```python
from build123d import *

# Parameters (mm, degrees)
BASE_PLATE_SKETCH_R = 7
BASE_PLATE_DEPTH    = 14
PIVOT_LUG_SKETCH_R  = 8
PIVOT_LUG_DEPTH     = 10


with BuildPart() as part:
    # Base Plate Sketch → Base Plate (new body)
    with BuildSketch(Plane.XY):
        with BuildLine():
            Line((-61, 29), (61, 29))
            ThreePointArc((61, 29), (64.535533906, 27.535533906), (66, 24))
            Line((66, 24), (66, -24))
            ThreePointArc((66, -24), (64.535533906, -27.535533906), (61, -29))
            Line((61, -29), (-61, -29))
            ThreePointArc((-61, -29), (-64.535533906, -27.535533906), (-66, -24))
            Line((-66, -24), (-66, 24))
            ThreePointArc((-66, 24), (-64.535533906, 27.535533906), (-61, 29))
        make_face()
        with Locations((-50, 0)):
            Circle(BASE_PLATE_SKETCH_R, mode=Mode.SUBTRACT)
        with Locations(Location((50, 0, 0), (0, 0, 180))):
            Circle(BASE_PLATE_SKETCH_R, mode=Mode.SUBTRACT)
    extrude(amount=BASE_PLATE_DEPTH)

    # Pivot Lug Sketch → Pivot Lug (add)
    with BuildSketch(Plane(origin=(0, 16, 0), x_dir=(1, 0, 0), z_dir=(0, 1, 0))):
        with BuildLine():
            Line((-37.5, 0), (37.5, 0))
            Line((37.5, 0), (18.575020612, 47.414081823))
            ThreePointArc((18.575020612, 47.414081823), (0, 60), (-18.575020612, 47.414081823))
            Line((-18.575020612, 47.414081823), (-37.5, 0))
        make_face()
        with Locations(Location((0, 40, 0), (0, 0, 270))):
            Circle(PIVOT_LUG_SKETCH_R, mode=Mode.SUBTRACT)
    pivot_lug = extrude(amount=PIVOT_LUG_DEPTH)

    # Pivot Lug Mirror: Pivot Lug across plane
    add(pivot_lug.mirror(Plane.ZX))


solid = part.part
```
The model under review builds one solid part; all positions refer to its coordinate system, in mm. A direction names the side the tool comes from. Give positions to 0.01 mm unless a question says otherwise; leave off trailing zeros. Write each loop counter-clockwise with the first axis right and the second up, starting at its lowest first coordinate (ties: lowest second). Pieces come first, ordered by that corner, then holes. Notation, with made-up numbers: (53.5, 88.5) - (58.5, 88.5) arc R19 cw to (58.5, 116.5) - close; hole circle Ø5 at (78, 18.5). An arc over 180 degrees is marked (long way). Answer in a Markdown table with one row per item. Add a question column.
1. Wall thickness on line 1 along Y through (x, z) = (-1.5, -51.5); line 2 along Z through (x, y) = (-2.5, 8.5); line 3 along X through (y, z) = (22, -40): over which ranges is each line inside the solid? List them lowest first. Write a range as [from, to].
2. Tool access review of faces 4 (the flat face through (-1, 16, -24)), 5 (the cylindrical face through (-65, 27, 7)): name each direction out of +Z, -Z, +X, -X, +Y, -Y from which nothing blocks a thin tool from reaching the whole face with its end or side.
3. We need section B-B on x = -50. Write out the cut boundary in (y, z).
4. We need section C-C on y = 0. Write out the cut boundary in (x, z), then the cut area to 3 significant figures.
5. Draft analysis for pull direction X (two halves, no side actions). For faces 1 (the cylindrical face through (-4.868, 20.93, -46.349)), 2 (the flat face through (-1, -26, -24)), 3 (the flat face through (28.17, 20.93, -23.38)), state which applies: +X half, -X half, draft (parallel to the pull), parting line (faces both ways), or undercut.
6. We need section A-A on z = 3. Write out the cut boundary in (x, y).
7. We need section D-D on x = 0. Write out the cut boundary in (y, z), then the cut area to 3 significant figures.
8. Insertion check: P1, Ø18.5, axis at x = 0, z = -40, coming from the +Y side; P2, Ø8, axis at x = -20.5, y = -16, coming from the -Z side; P3, Ø2, axis at y = -15.5, z = -37, coming from the +X side. Each pin has a flat end and moves straight along its axis. Give the tip position at first contact, or say it passes through.
Ans:
| question | item | result |
|---|---|---|
| 1 | line 1 | y = [-26, -16], [16, 26] |
| 1 | line 2 | z = [0, 14] |
| 1 | line 3 | x = [-21.53, -8], [8, 21.53] |
| 2 | face 4 | -Z, +X, -X |
| 2 | face 5 | +Z, -Z, -X, +Y |
| 3 | outline | (-29, 0) - (-7, 0) - (-7, 14) - (-29, 14) - close; (7, 0) - (29, 0) - (29, 14) - (7, 14) - close |
| 4 | outline | (-66, 0) - (-57, 0) - (-57, 14) - (-66, 14) - close; (-43, 0) - (43, 0) - (43, 14) - (-43, 14) - close; (57, 0) - (66, 0) - (66, 14) - (57, 14) - close |
| 4 | area | 1,460 mm^2 |
| 5 | face 1 | undercut |
| 5 | face 2 | draft |
| 5 | face 3 | +X half |
| 6 | outline | (-66, -24) arc R5 ccw to (-61, -29) - (61, -29) arc R5 ccw to (66, -24) - (66, 24) arc R5 ccw to (61, 29) - (-61, 29) arc R5 ccw to (-66, 24) - close; hole circle Ø14 at (-50, 0); hole circle Ø14 at (50, 0) |
| 7 | outline | (-29, 0) - (-26, 0) - (-26, -32) - (-16, -32) - (-16, 0) - (16, 0) - (16, -32) - (26, -32) - (26, 0) - (29, 0) - (29, 14) - (-29, 14) - close; (-26, -60) - (-16, -60) - (-16, -48) - (-26, -48) - close; (16, -60) - (26, -60) - (26, -48) - (16, -48) - close |
| 7 | area | 1,690 mm^2 |
| 8 | P1 | stops at y = 26 |
| 8 | P2 | stops at z = -51.3 |
| 8 | P3 | stops at x = 23.08 |
